from build123d import *

# Parameters (mm, degrees)
SKETCH1_W                                           = 160
SKETCH1_H                                           = 60
BOSS_EXTRUDE1_DEPTH                                 = 5
CBORE_FOR_M6_HEX_SOCKET_HEAD_CAP_SCREW1_D           = 6.6
CBORE_FOR_M6_HEX_SOCKET_HEAD_CAP_SCREW1_CBORE_D     = 11
CBORE_FOR_M6_HEX_SOCKET_HEAD_CAP_SCREW1_CBORE_DEPTH = 6.4
CHAMFER1_SIZE                                       = 5
M6_TAPPED_HOLE1_D                                   = 5
M6_TAPPED_HOLE1_DEPTH                               = 11
M6_TAPPED_HOLE1_TIP                                 = 1.502151548


with BuildPart() as part:
    # Sketch1 → Boss-Extrude1 (new, symmetric)
    with BuildSketch(Plane.XY):
        Rectangle(SKETCH1_W, SKETCH1_H)
    extrude(amount=BOSS_EXTRUDE1_DEPTH, both=True)

    # CBORE for M6 Hex Socket Head Cap Screw1 (through all)
    with Locations(Plane.XY.offset(5)):
        with Locations((35, -16), (65, -16), (65, 16), (35, 16)):
            CounterBoreHole(CBORE_FOR_M6_HEX_SOCKET_HEAD_CAP_SCREW1_D / 2, CBORE_FOR_M6_HEX_SOCKET_HEAD_CAP_SCREW1_CBORE_D / 2, CBORE_FOR_M6_HEX_SOCKET_HEAD_CAP_SCREW1_CBORE_DEPTH)

    # Chamfer1
    chamfer1_edges = [part.edges().sort_by_distance(p)[0] for p in [
        (80, -30, 0),
        (80, 30, 0),
    ]]
    chamfer(chamfer1_edges, length=CHAMFER1_SIZE)

    # M6 Tapped Hole1
    with Locations(Plane.ZY.offset(80)):
        with Locations((0, 18), (0, 0), (0, -18)):
            Hole(M6_TAPPED_HOLE1_D / 2, depth=M6_TAPPED_HOLE1_DEPTH)
            with Locations((0, 0, -(M6_TAPPED_HOLE1_DEPTH + M6_TAPPED_HOLE1_TIP / 2))):  # 118° drill point
                Cone(0, M6_TAPPED_HOLE1_D / 2, M6_TAPPED_HOLE1_TIP, mode=Mode.SUBTRACT)


solid = part.part
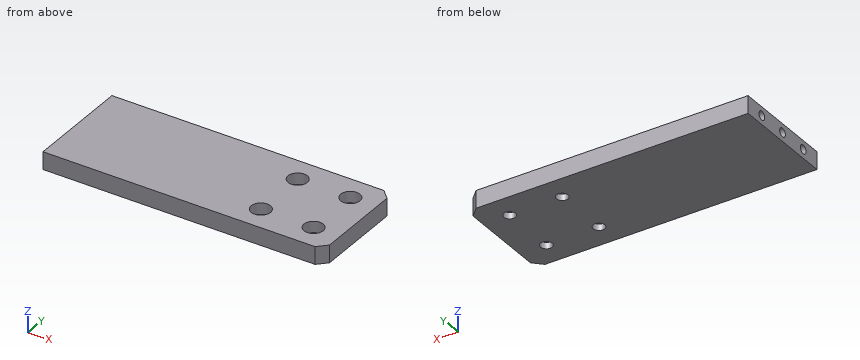
Input: part model. Units: mm. Frame: model coordinates. Give positions to 0.01 mm unless a question says otherwise; leave off trailing zeros. Loops run counter-clockwise (first coordinate to the right, second up) from the corner with the lowest first, then second, coordinate; pieces in that order, holes last. Notation, with made-up numbers: (-5.5, -2.5) - (7.5, -2.5) arc R22 cw to (7.5, 23.5) - close; hole circle Ø8 at (38, 13.5). An arc over 180 degrees is marked (long way). Use CSV: the item, a comma, the result in double quotes. Start each with the question number.
Item 1: Section A-A on x = 65. Return loops of the section in (y, z).
Item 2: Line query: line 1 (X direction, y = -15.5, z = 4); line 2 (Y direction, x = -71, z = 0); line 3 (Y direction, x = 35, z = 2). Output: solid intervals per line, ascending.
Item 3: Contact query for flat-ended pins moving along their axis: P1, Ø3.5, axis at x = 63, y = -18.5, coming from the +Z side; P2, Ø4, axis at x = 65, y = -16, coming from the -Z side; P3, Ø6, axis at y = 18, z = 0, coming from the -X side. Output: stop coordinate, or through.
Ans:
1,outline,"(-30, -5) - (-19.3, -5) - (-19.3, -1.4) - (-21.5, -1.4) - (-21.5, 5) - (-30, 5) - close; (-12.7, -5) - (12.7, -5) - (12.7, -1.4) - (10.5, -1.4) - (10.5, 5) - (-10.5, 5) - (-10.5, -1.4) - (-12.7, -1.4) - close; (19.3, -5) - (30, -5) - (30, 5) - (21.5, 5) - (21.5, -1.4) - (19.3, -1.4) - close"
2,line 1,"x = -80 to 29.52, 40.48 to 59.52, 70.48 to 80"
2,line 2,"y = -30 to -20.5, -15.5 to -2.5, 2.5 to 15.5, 20.5 to 30"
2,line 3,"y = -30 to -21.5, -10.5 to 10.5, 21.5 to 30"
3,P1,"stops at z = -1.4"
3,P2,"passes through"
3,P3,"stops at x = -80"
